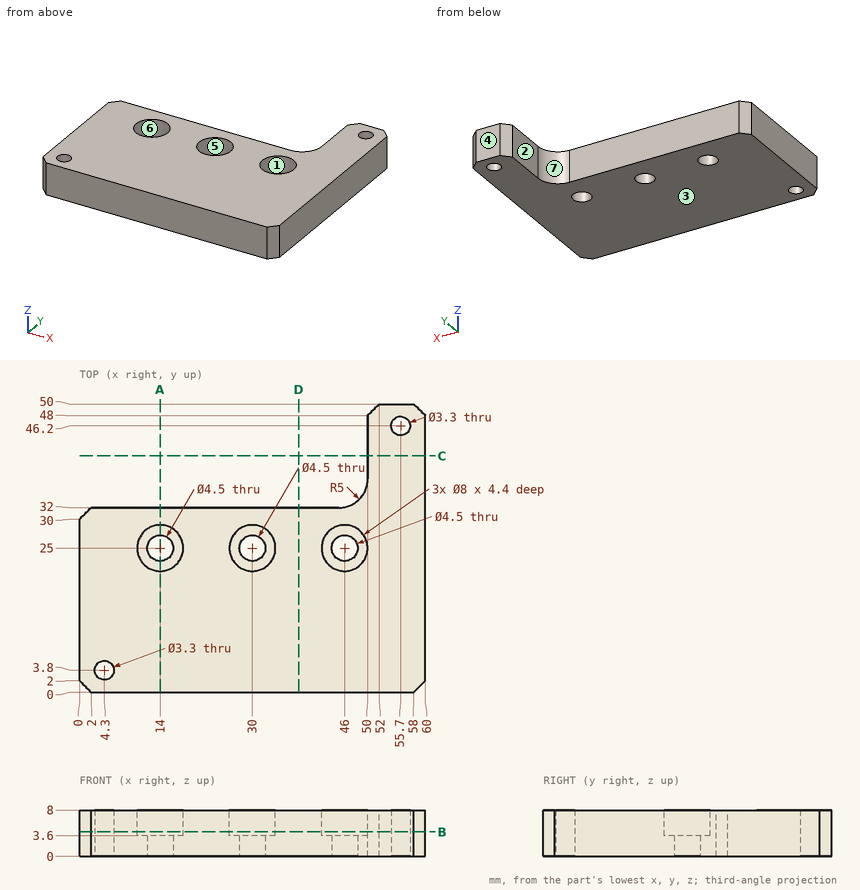
Study the drawing (mm; zero at the part's minimum x, y, z) and answer. A direction names the side the tool comes from. Give positions to 0.01 mm unless a question says otherwise; leave off trailing zeros. Loops run counter-clockwise (first coordinate to the right, second up) from the corner with the lowest first, then second, coordinate; pieces in that order, holes last. Notation, with made-up numbers: (34.25, -4) -> (62.25, -4) arc R26 cw to (62.25, 21) -> close; hole circle Ø1 at (-11, 59.25). An arc over 180 degrees is marked (long way). Write item = value, one per line. Start each with the question number.
(1) Find section C-C on y = 41. Give the vertices of the cut face in (x, z), and give its area (3 significant figures).
(2) Find the intervals of material crossed by probe 1 along X at (y, z) = (4, 5.75); probe 2 along Y at (x, z) = (14, 0.85); probe 3 along Y at (x, z) = (21, 0.5), in increasing order. Write a range as from..to.
(3) The mould has two halves that part along X. Classify the marked faces 4, 5, 6 and 7: +X half, -X half, draft (parallel to the pull), parting line (faces both ways), or undercut.
(4) Find section D-D on x = 38. Give the vertices of the cut face in (y, z), and give its area (3 significant figures).
(5) Given pin 1 Ø4 at (y, z) = (44.5, 5.5) entering from -X; pin 2 Ø4 at (x, z) = (13, 6) entering from +Y; pin 3 Ø13 at (x, y) = (14, 25) entering from +Z; pin 4 Ø2.5 at (x, y) = (44.5, 25) entering from +Z, each flat-ended and moving along its own axis, determine where each tip first touches the part or whether it passes through.
(6) Which of the six approach directions +Z, -Z, +X, -X, +Y, -Y give full straight-line access (tool end or side, diameter ignored) to the marked faces 1, 2 and 3?
(7) Find section B-B on z = 4.25. Give the vertices of the cut face in (x, y).
(8) Find section A-A on x = 14. Give the vertices of the cut face in (y, z).
From the geometry:
q1.outline = (50, 0) -> (60, 0) -> (60, 8) -> (50, 8) -> close
q1.area = 80.0 mm^2
q2.probe_1 = 0..2.66, 5.94..60
q2.probe_2 = 0..22.75, 27.25..32
q2.probe_3 = 0..32
q3.face_4 = draft
q3.face_5 = undercut
q3.face_6 = undercut
q3.face_7 = -X half
q4.outline = (0, 0) -> (32, 0) -> (32, 8) -> (0, 8) -> close
q4.area = 256 mm^2
q5.pin_1 = 50
q5.pin_2 = 32
q5.pin_3 = 8
q5.pin_4 = 3.6
q6.face_1 = +Z
q6.face_2 = +Z, -Z, -X, +Y
q6.face_3 = -Z, +X, -X, +Y, -Y
q7.outline = (0, 2) -> (2, 0) -> (58, 0) -> (60, 2) -> (60, 48) -> (58, 50) -> (52, 50) -> (50, 48) -> (50, 37) arc R5 cw to (45, 32) -> (2, 32) -> (0, 30) -> close; hole circle Ø3.3 at (4.3, 3.8); hole circle Ø8 at (14, 25); hole circle Ø8 at (30, 25); hole circle Ø8 at (46, 25); hole circle Ø3.3 at (55.7, 46.2)
q8.outline = (0, 0) -> (22.75, 0) -> (22.75, 3.6) -> (21, 3.6) -> (21, 8) -> (0, 8) -> close; (27.25, 0) -> (32, 0) -> (32, 8) -> (29, 8) -> (29, 3.6) -> (27.25, 3.6) -> close
